Read the model definition and answer for the solid it produces. Units are mm, in the model's axes. Face numbers are marked on the shaded views. A direction names the side the tool comes from. Give positions to 0.01 mm unless a question says otherwise; leave off trailing zeros. Order: outer loops, then holes, each group sorted by start corner. A loop starts at its lowest first (then second) coordinate and runs counter-clockwise, first axis right, second up. Notation, with made-up numbers: (-35.75, 13.5) -> (2.25, 13.5) arc R28 cw to (2.25, 43.5) -> close; hole circle Ø9 at (78.25, 7). An arc over 180 degrees is marked (long way). Use one line per item in the form item = value.
```python
from build123d import *

# Parameters (mm, degrees)
SKETCH_1_W                = 103
SKETCH_1_H                = 100
EXTRUDE_1_DEPTH           = 10
SKETCH_9_W                = 15.5
SKETCH_9_H                = 88
CUT_EXTRUDE_4_DEPTH       = 144.906219463
HOLE_WIZARD_6_5_6_5_1_D   = 6.5
SKETCH_12_R               = 17.5
CUT_EXTRUDE_5_DEPTH       = 144.906219463
FILLET_1_R                = 10
HOLE_WIZARD_5_0_5_1_D     = 5
HOLE_WIZARD_5_0_5_1_DEPTH = 10
HOLE_WIZARD_5_0_5_1_TIP   = 1.502151548
FILLET_2_R                = 2
SKETCH_20_W               = 140.430498758
SKETCH_20_H               = 45.630669844
CUT_EXTRUDE_6_DEPTH       = 97
HOLE_WIZARD_1_D           = 4.4
HOLE_WIZARD_1_CBORE_D     = 8
HOLE_WIZARD_1_CBORE_DEPTH = 5
HOLE_WIZARD_M6_2_D        = 5
SKETCH_28_W               = 143.680703706
SKETCH_28_H               = 10.15
CUT_EXTRUDE_7_DEPTH       = 2


with BuildPart() as part:
    # 草图1 → 凸台-拉伸1 (new body)
    with BuildSketch(Plane(origin=(0, 0, 0), x_dir=(1, 0, 0), z_dir=(0, 1, 0))):
        with Locations((51.5, -50)):
            Rectangle(SKETCH_1_W, SKETCH_1_H)
    extrude(amount=EXTRUDE_1_DEPTH)

    # 草图9 → 切除-拉伸4 (cut, through all)
    with BuildSketch(Plane(origin=(0, 10, 0), x_dir=(1, 0, 0), z_dir=(0, 1, 0))):
        with Locations((7.75, -56)):
            Rectangle(SKETCH_9_W, SKETCH_9_H)
        with Locations((95.25, -56)):
            Rectangle(SKETCH_9_W, SKETCH_9_H)
    extrude(amount=-CUT_EXTRUDE_4_DEPTH, mode=Mode.SUBTRACT)

    # Ø6.5 (6.5) 直径孔1 (through all)
    with Locations(Plane.XY.offset(12)):
        with Locations((6, 5), (97, 5)):
            Hole(HOLE_WIZARD_6_5_6_5_1_D / 2)

    # 草图12 → 切除-拉伸5 (cut, through all)
    with BuildSketch(Plane(origin=(0, 10, 0), x_dir=(1, 0, 0), z_dir=(0, 1, 0))):
        with Locations(Location((51.5, -68, 0), (0, 0, 270))):
            Circle(SKETCH_12_R)
    extrude(amount=-CUT_EXTRUDE_5_DEPTH, mode=Mode.SUBTRACT)

    # 圆角1
    fillet_1_edges = [part.edges().sort_by_distance(p)[0] for p in [
        (15.5, 5, 100),
        (87.5, 5, 100),
    ]]
    fillet(fillet_1_edges, radius=FILLET_1_R)

    # Ø5.0 (5) 直径孔1
    with Locations(Plane(origin=(0, 0, 0), x_dir=(-1, 0, 0), z_dir=(0, 0, -1))):
        with Locations((-71.5, 5), (-31.5, 5)):
            Hole(HOLE_WIZARD_5_0_5_1_D / 2, depth=HOLE_WIZARD_5_0_5_1_DEPTH)
            with Locations((0, 0, -(HOLE_WIZARD_5_0_5_1_DEPTH + HOLE_WIZARD_5_0_5_1_TIP / 2))):  # 118° drill point
                Cone(0, HOLE_WIZARD_5_0_5_1_D / 2, HOLE_WIZARD_5_0_5_1_TIP, mode=Mode.SUBTRACT)

    # 圆角2
    fillet_2_edges = [part.edges().sort_by_distance(p)[0] for p in [
        (15.5, 5, 12),
        (87.5, 5, 12),
    ]]
    fillet(fillet_2_edges, radius=FILLET_2_R)

    # 草图20 → 切除-拉伸6 (cut)
    with BuildSketch(Plane(origin=(0, 10, 0), x_dir=(1, 0, 0), z_dir=(0, 1, 0))):
        with Locations((42.090220098, -13.184665078)):
            Rectangle(SKETCH_20_W, SKETCH_20_H)
    extrude(amount=-CUT_EXTRUDE_6_DEPTH, mode=Mode.SUBTRACT)

    # 打孔尺寸(%根据)内六角圆柱头螺钉的类型1 (through all)
    with Locations(Plane(origin=(0, 10, 0), x_dir=(1, 0, 0), z_dir=(0, 1, 0))):
        with Locations((21.5, -48), (81.5, -48)):
            CounterBoreHole(HOLE_WIZARD_1_D / 2, HOLE_WIZARD_1_CBORE_D / 2, HOLE_WIZARD_1_CBORE_DEPTH)

    # M6 螺纹孔2 (through all)
    with Locations(Plane(origin=(0, 10, 0), x_dir=(1, 0, 0), z_dir=(0, 1, 0))):
        with Locations((26.5, -43), (26.5, -93), (76.5, -93), (76.5, -43)):
            Hole(HOLE_WIZARD_M6_2_D / 2)

    # 草图28 → 切除-拉伸7 (cut)
    with BuildSketch(Plane.XZ):
        with Locations((21.5, 48)):
            Rectangle(SKETCH_28_W, SKETCH_28_H)
    extrude(amount=-CUT_EXTRUDE_7_DEPTH, mode=Mode.SUBTRACT)


solid = part.part
```
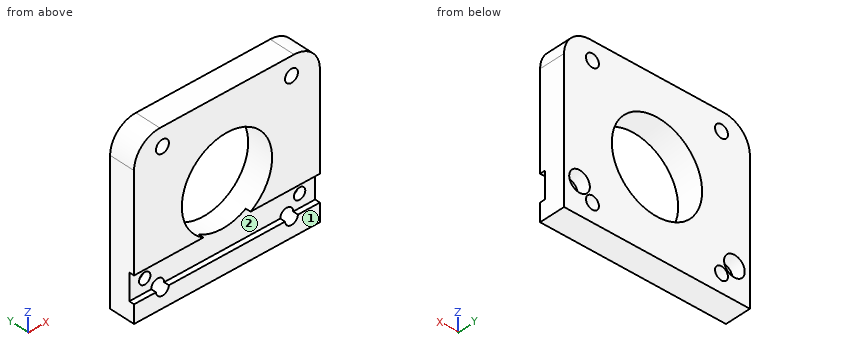
Item 1: Straight lines are drawn through the part: L1, parallel to X at y = 4.75, z = 43; L2, parallel to X at y = 8.1, z = 48; L3, parallel to Z at x = 76.5, y = 5.75. For each, find the intervals that lie inside material, in ascending order. Write a range as from..to.
Checks:
L1 = 15.5..24, 29..74, 79..87.5
L2 = 15.5..17.5, 25.5..77.5, 85.5..87.5
L3 = 36..40.5, 45.5..90.5, 95.5..100
Item 2: The part is cut by section C-C on z = 68. Give the vertices of the cut face in (x, y).
Checks:
outline = (15.5, 0) -> (34, 0) -> (34, 10) -> (15.5, 10) -> close; (69, 0) -> (87.5, 0) -> (87.5, 10) -> (69, 10) -> close
Item 3: The part is cut by section B-B on y = 6.5. Give the vertices of the cut face in (x, z).
Checks:
outline = (15.5, 36) -> (87.5, 36) -> (87.5, 90) arc R10 ccw to (77.5, 100) -> (25.5, 100) arc R10 ccw to (15.5, 90) -> close; hole circle Ø8 at (21.5, 48); hole circle Ø5 at (26.5, 43); hole circle Ø5 at (26.5, 93); hole circle Ø35 at (51.5, 68); hole circle Ø5 at (76.5, 43); hole circle Ø5 at (76.5, 93); hole circle Ø8 at (81.5, 48)
Item 4: Which of the six approach directions +Z, -Z, +X, -X, +Y, -Y give full straight-line access (tool end or side, diameter ignored) to the marked faces 1 and 2?
Checks:
face_1 = +Z, -Z, +X, -X, -Y
face_2 = +X, -X, -Y
Item 5: The part is cut by section A-A on x = 26.5. Give the vertices of the cut face in (y, z) (3 decimals), and give its area (3 significant figures).
Checks:
outline = (0, 36) -> (10, 36) -> (10, 40.5) -> (0, 40.5) -> close; (0, 53.075) -> (2, 53.075) -> (2, 45.5) -> (10, 45.5) -> (10, 90.5) -> (0, 90.5) -> close; (0, 95.5) -> (10, 95.5) -> (10, 100) -> (0, 100) -> close
area = 525 mm²
Item 6: Given pin 1 Ø5.5 at (x, z) = (81.5, 48) entering from -Y; pin 2 Ø2.5 at (x, z) = (19.5, 48) entering from +Y; pin 3 Ø9 at (x, z) = (81.5, 48) entering from +Y; pin 4 Ø1 at (x, y) = (19, 1.5) entering from +Z, each flat-ended and moving along its own axis, determine where each tip first touches the part or whether it passes through.
Checks:
pin_1 = 2
pin_2 = 5
pin_3 = 10
pin_4 = 98
Item 7: The part is cut by section D-D on x = 81.5. Give the vertices of the cut face in (y, z) (3 decimals).
Checks:
outline = (0, 36) -> (10, 36) -> (10, 44) -> (5, 44) -> (5, 45.8) -> (2, 45.8) -> (2, 42.925) -> (0, 42.925) -> close; (0, 53.075) -> (2, 53.075) -> (2, 50.2) -> (5, 50.2) -> (5, 52) -> (10, 52) -> (10, 99.165) -> (0, 99.165) -> close
